Source: CAD feature listing. Evaluate the final solid. Frame: model axes, mm. A direction names the side the tool comes from. Coordinates: 2 decimals unless noted, no trailing zeros. Write each loop counter-clockwise with the first axis right and the second up, starting at its lowest first coordinate (ties: lowest second). Pieces come first, ordered by that corner, then holes. Notation, with made-up numbers: (8, 57) -> (15, 57) arc R37 cw to (15, 94) -> close; hole circle Ø4 at (6.5, 69.25). An arc over 180 degrees is marked (long way). Write item = value, one per line.
from build123d import *

# Parameters (mm, degrees)
SKETCH4_R          = 16
CUT_EXTRUDE2_DEPTH = 120


with BuildPart() as part:
    # Sketch1 → Revolve1 (revolve)
    with BuildSketch(Plane.XY, mode=Mode.PRIVATE) as revolve1_sk:
        Polygon((0, 21.901923789), (4.5, 24.5), (10.25, 16.5), (13, 16.5), (13, 0), (-13, 0), (-13, 16.5), (-10.25, 16.5), (-4.5, 24.5), align=None)
    revolve(revolve1_sk.sketch.rotate(Axis((-38.0976844, 0, 0), (1, 0, 0)), 180), axis=Axis((-38.0976844, 0, 0), (1, 0, 0)))

    # Sketch3 → Cut-Revolve1 (revolve, cut)
    with BuildSketch(Plane.XY):
        Polygon((4.216204142, 23.181449847), (0, 20.74722325), (-4.216204142, 23.181449847), (-9.737246219, 15.5), (-12, 15.5), (-12, 1), (-12, 0), (12, 0), (12, 1), (12, 15.5), (9.737246219, 15.5), align=None)
    revolve(axis=Axis((12, 0, 0), (-1, 0, 0)), mode=Mode.SUBTRACT)

    # Sketch4 → Cut-Extrude2 (cut)
    with BuildSketch(Plane(origin=(13, 0, 0), x_dir=(0, 0, -1), z_dir=(1, 0, 0))):
        with Locations(Location((0, 0, 0), (0, 0, 90))):
            Circle(SKETCH4_R)
    extrude(amount=-CUT_EXTRUDE2_DEPTH, mode=Mode.SUBTRACT)


solid = part.part
1) Cut plane D-D, the plane x = -3. Output: boundary loops of the cut face in (y, z), and give its area (3 significant figures).
Answer block:
outline = circle Ø47.27 at (0, 0); hole circle Ø44.96 at (0, 0)
area = 167 mm2
2) Reachability of faces 1 (the conical face through (-0.218, 17.481, 13.404)), 2 (the cylindrical face through (-11.16, -3.47, -15.62)), 3 (the cylindrical face through (11.644, -15.738, -4.956)), 4 (the flat face through (-13, -16, -3)), 5 (the cylindrical face through (-11.606, -15.738, -4.956)) from +Z, -Z, +X, -X, +Y, -Y: full face, straight path, thin tool, end or side. Return the list, or none.
Answer block:
face_1 = none
face_2 = +X, -X
face_3 = +X
face_4 = +Z, -Z, -X, +Y, -Y
face_5 = -X
3) Material intervals for probe 1 along X at (y, z) = (20, -6); probe 2 along Z at (x, y) = (11.7, 0); probe 3 along X at (y, z) = (-7, 21), sorted ascending. Write a range as [from, to].
Answer block:
probe_1 = [-7.1, -5.87], [-0.23, 0.23], [5.87, 7.1]
probe_2 = [-16.5, -16], [16, 16.5]
probe_3 = [-6.2, -4.97], [-2.41, -0.41], [0.41, 2.41], [4.97, 6.2]
4) Cut plane A-A, the plane y = 0. Output: boundary loops of the cut face in (x, z), and give its area (3 significant figures).
Answer block:
outline = (-13, -16.5) -> (-10.25, -16.5) -> (-4.5, -24.5) -> (0, -21.9) -> (4.5, -24.5) -> (10.25, -16.5) -> (13, -16.5) -> (13, -16) -> (9.38, -16) -> (4.22, -23.18) -> (0, -20.75) -> (-4.22, -23.18) -> (-9.38, -16) -> (-13, -16) -> close; (-13, 16) -> (-9.38, 16) -> (-4.22, 23.18) -> (0, 20.75) -> (4.22, 23.18) -> (9.38, 16) -> (13, 16) -> (13, 16.5) -> (10.25, 16.5) -> (4.5, 24.5) -> (0, 21.9) -> (-4.5, 24.5) -> (-10.25, 16.5) -> (-13, 16.5) -> close
area = 63.9 mm2
5) First-contact query: pin 1 Ø2 at (y, z) = (17.5, 2.5) entering from -X; pin 2 Ø5 at (y, z) = (-7, -9.5) entering from +X; pin 3 Ø10 at (y, z) = (19.5, -2) entering from +X; pin 4 Ø2 at (x, y) = (-3, -16) entering from -Z. Flat tips, straight axial feed; report the tip coordinate or a pass-through.
Answer block:
pin_1 = -10.12
pin_2 = through
pin_3 = 13
pin_4 = -18.55
6) Cut plane C-C, the plane x = 11. Output: boundary loops of the cut face in (y, z), and give its area (3 significant figures).
Answer block:
outline = circle Ø33 at (0, 0); hole circle Ø32 at (0, 0)
area = 51.1 mm2
7) Pull-direction query (Y, two-part tool) for faces 6 (the flat face through (13, 3, -16)), 7 (the conical face through (9.97, -16.11, -5.07)), 8 (the conical face through (9.055, -3.566, 16.058)); classes: +Y half, -Y half, draft (parallel to the pull), parting line (faces both ways), or undercut.
Answer block:
face_6 = draft
face_7 = parting line
face_8 = undercut
